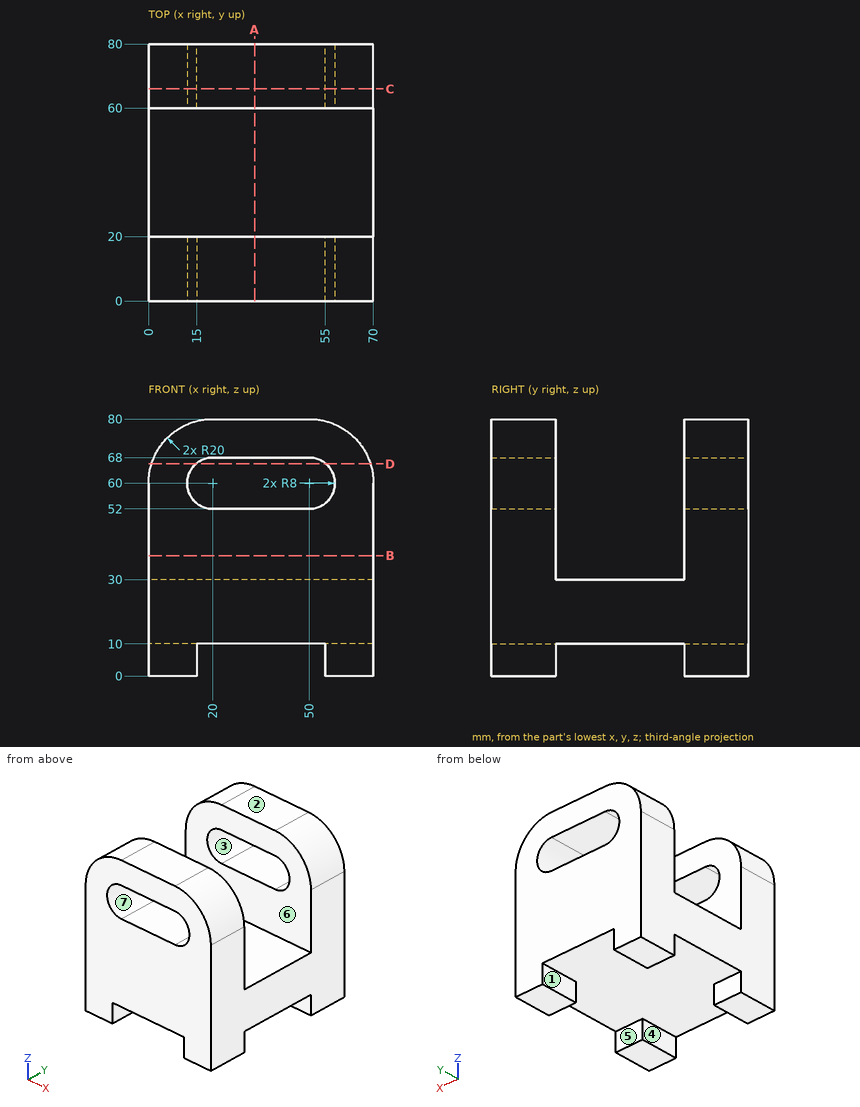
Study the drawing (mm; zero at the part's minimum x, y, z) and answer. A direction names the side the tool comes from. Coordinates: 2 decimals unless noted, no trailing zeros. Write each loop counter-clockwise with the first axis right and the second up, starting at its lowest first coordinate (ties: lowest second). Pieces come first, ordered by that corner, then holes. Notation, with made-up numbers: (20, 17) - (24, 17) arc R19 cw to (24, 28) - close; hole circle Ø6 at (1, 16.5). An arc over 180 degrees is marked (long way). Put each result on its own line as item: value.
1. The part is cut by section A-A on x = 33. Give the vertices of the cut face in (y, z), plus the area to 3 significant figures.
Answer sheet:
outline: (0, 10) - (80, 10) - (80, 52) - (60, 52) - (60, 30) - (20, 30) - (20, 52) - (0, 52) - close; (0, 68) - (20, 68) - (20, 80) - (0, 80) - close; (60, 68) - (80, 68) - (80, 80) - (60, 80) - close
area: 2,960 mm^2
2. The part is cut by section D-D on z = 66. Give the vertices of the cut face in (x, y), plus the area to 3 significant figures.
Answer sheet:
outline: (0.92, 0) - (14.71, 0) - (14.71, 20) - (0.92, 20) - close; (0.92, 60) - (14.71, 60) - (14.71, 80) - (0.92, 80) - close; (55.29, 0) - (69.08, 0) - (69.08, 20) - (55.29, 20) - close; (55.29, 60) - (69.08, 60) - (69.08, 80) - (55.29, 80) - close
area: 1,100 mm^2
3. A tool of negligible diameter and unlimited length cuts with its end or side. For the marked faces 4, 5, 6 and 7, from which of +Z, -Z, +X, -X, +Y, -Y can it reach the whole face along a straight path? Write none if from no direction.
Answer sheet:
face 4: -Z, +Y, -Y
face 5: -Z, +X, -X
face 6: +Z, +X, -X
face 7: +Y, -Y
4. Find the intervals of material crossed by line 1 along Y through (x, z) = (64.5, 54.5); line 2 along X through (y, z) = (61.5, 59.5); line 3 along X through (y, z) = (70.5, 7), in increasing order. Write a range as from..to.
Answer sheet:
line 1: y = 0..20, 60..80
line 2: x = 0..12.02, 57.98..70
line 3: x = 0..15, 55..70
5. Flat-ended cylindrical pins translate along their axes: pin 1 Ø16 at (x, y) = (40.5, 6) entering from -Z; pin 2 Ø4 at (x, y) = (8.5, 52.5) entering from +Z. Find the tip coordinate at first contact, or state that the pin passes through.
Answer sheet:
pin 1: stops at z = 10
pin 2: stops at z = 30
6. The part is cut by section B-B on z = 37.5. Give the vertices of the cut face in (x, y), plus the area to 3 significant figures.
Answer sheet:
outline: (0, 0) - (70, 0) - (70, 20) - (0, 20) - close; (0, 60) - (70, 60) - (70, 80) - (0, 80) - close
area: 2,800 mm^2
7. Determine the mould class of the marked faces 1, 2 and 3 for opening direction Z: pulls with the +Z half, pulls with the -Z half, needs draft (parallel to the pull), parting line crosses it, or undercut.
Answer sheet:
face 1: needs draft
face 2: pulls with the +Z half
face 3: undercut
8. The part is cut by section C-C on y = 66. Give the vertices of the cut face in (x, z), plus the area to 3 significant figures.
Answer sheet:
outline: (0, 0) - (15, 0) - (15, 10) - (55, 10) - (55, 0) - (70, 0) - (70, 60) arc R20 ccw to (50, 80) - (20, 80) arc R20 ccw to (0, 60) - close; hole (20, 52) - (50, 52) arc R8 ccw to (50, 68) - (20, 68) arc R8 ccw to start
area: 4,350 mm^2
